from build123d import *

# Parameters (mm, degrees)
SKETCH_1_W                = 192
SKETCH_1_H                = 200
EXTRUDE_1_DEPTH           = 7.5
CHAMFER_1_SIZE            = 1
HOLE_WIZARD_1_D           = 6.6
HOLE_WIZARD_1_CBORE_D     = 11
HOLE_WIZARD_1_CBORE_DEPTH = 6.8
SKETCH_7_R                = 62
CUT_EXTRUDE_1_DEPTH       = 15
HOLE_WIZARD_M6_1_D        = 5


with BuildPart() as part:
    # 草图1 → 凸台-拉伸1 (new, symmetric)
    with BuildSketch(Plane(origin=(0, 0, 0), x_dir=(1, 0, 0), z_dir=(0, 1, 0))):
        Rectangle(SKETCH_1_W, SKETCH_1_H)
    extrude(amount=EXTRUDE_1_DEPTH, both=True)

    # 倒角1
    chamfer_1_edges = [part.edges().sort_by_distance(p)[0] for p in [
        (96, 0, 100),
        (-96, 0, 100),
        (-96, 0, -100),
        (96, 0, -100),
    ]]
    chamfer(chamfer_1_edges, length=CHAMFER_1_SIZE)

    # 打孔尺寸(%根据)内六角圆柱头螺钉的类型1 (through all)
    with Locations(Plane(origin=(0, -7.5, 0), x_dir=(-1, 0, 0), z_dir=(0, -1, 0))):
        with Locations((90, -90), (90, -30), (-90, -30), (-90, -90), (-90, 90), (-90, 30), (90, 30), (90, 90)):
            CounterBoreHole(HOLE_WIZARD_1_D / 2, HOLE_WIZARD_1_CBORE_D / 2, HOLE_WIZARD_1_CBORE_DEPTH)

    # 草图7 → 切除-拉伸1 (cut)
    with BuildSketch(Plane(origin=(0, 7.5, 0), x_dir=(1, 0, 0), z_dir=(0, 1, 0))):
        with Locations(Location((0, 0, 0), (0, 0, 270))):
            Circle(SKETCH_7_R)
    extrude(amount=-CUT_EXTRUDE_1_DEPTH, mode=Mode.SUBTRACT)

    # M6 螺纹孔1 (through all)
    with Locations(Plane(origin=(0, -7.5, 0), x_dir=(-1, 0, 0), z_dir=(0, -1, 0))):
        with Locations((67.5, 0), (62.361868445, -25.831131685), (47.72970773, -47.72970773), (25.831131685, -62.361868445), (0, -67.5), (-25.831131685, -62.361868445), (-47.72970773, -47.72970773), (-62.361868445, -25.831131685), (-67.5, 0), (-62.361868445, 25.831131685), (-47.72970773, 47.72970773), (-25.831131685, 62.361868445), (0, 67.5), (25.831131685, 62.361868445), (47.72970773, 47.72970773), (62.361868445, 25.831131685)):
            Hole(HOLE_WIZARD_M6_1_D / 2)


solid = part.part
Design review of the part built by this model. Coordinates are the model's own, in mm. A direction names the side the tool comes from. Coordinates: 2 decimals unless noted, no trailing zeros. Write each loop counter-clockwise with the first axis right and the second up, starting at its lowest first coordinate (ties: lowest second). Pieces come first, ordered by that corner, then holes. Notation, with made-up numbers: (44, -39.5) - (49, -39.5) arc R20 cw to (49, -19.5) - close; hole circle Ø11 at (32, 55). An arc over 180 degrees is marked (long way). Use one line per item in the form item = value.
Q1. Consider section B-B (z = 90). Write out the cut boundary in (x, y), plus the area to 3 significant figures.
Taken from the geometry:
outline = (-96, -7.5) - (-95.5, -7.5) - (-95.5, -0.7) - (-93.3, -0.7) - (-93.3, 7.5) - (-96, 7.5) - close; (-86.7, -0.7) - (-84.5, -0.7) - (-84.5, -7.5) - (84.5, -7.5) - (84.5, -0.7) - (86.7, -0.7) - (86.7, 7.5) - (-86.7, 7.5) - close; (93.3, -0.7) - (95.5, -0.7) - (95.5, -7.5) - (96, -7.5) - (96, 7.5) - (93.3, 7.5) - close
area = 2,620 mm^2
Q2. The part is to be moulded in two halves that separate along Z. For faces 1 (the flat face through (-1, 0, -100)), 2 (the flat face through (-44, 7.5, -46)), 3 (the cylindrical face through (-45.42, 0.11, -46.77)), say which applies: +Z half, -Z half, draft (parallel to the pull), parting line (faces both ways), or undercut.
Taken from the geometry:
face_1 = -Z half
face_2 = draft
face_3 = undercut
Q3. Insertion check: pin 1 Ø3.5 at (x, z) = (91, -92.5) entering from -Y. The pin has a flat end and moves straight along its axis. Give the tip position at first contact, or say it passes through.
Taken from the geometry:
pin_1 = -0.7
Q4. Consider section D-D (y = -4.75). Count the separate pieces of the cut face and the enclosed holes in it, plus the area to 3 significant figures.
Taken from the geometry:
separate_pieces = 1
enclosed_holes = 25
area = 25,200 mm^2
Q5. Machinability: for faces 4 (the cylindrical face through (94.05, -4.15, -93.72)), 5 (the cylindrical face through (86.7, 3.5, -30.1)), which of the approach directions +Z, -Z, +X, -X, +Y, -Y give a long, thin tool a straight path to every point of the face, cutting with its end or side? Answer none if there is none.
Taken from the geometry:
face_4 = -Y
face_5 = +Y, -Y
Q6. For probe 1 along Z at (x, y) = (-90, 5); probe 2 along X at (y, z) = (0.75, 67.5); probe 3 along X at (y, z) = (-5, -90), list the stretches that pass through material, from the lowest coordinate up.
Taken from the geometry:
probe_1 = -100 to -93.3, -86.7 to -33.3, -26.7 to 26.7, 33.3 to 86.7, 93.3 to 100
probe_2 = -96 to -2.5, 2.5 to 96
probe_3 = -96 to -95.5, -84.5 to 84.5, 95.5 to 96
Q7. Consider section A-A (x = 0). Write out the cut boundary in (y, z), plus the area to 3 significant figures.
Taken from the geometry:
outline = (-7.5, -100) - (7.5, -100) - (7.5, -70) - (-7.5, -70) - close; (-7.5, -65) - (7.5, -65) - (7.5, -62) - (-7.5, -62) - close; (-7.5, 62) - (7.5, 62) - (7.5, 65) - (-7.5, 65) - close; (-7.5, 70) - (7.5, 70) - (7.5, 100) - (-7.5, 100) - close
area = 990 mm^2
Q8. Consider section C-C (x = -67.5). Write out the cut boundary in (y, z).
Taken from the geometry:
outline = (-7.5, -100) - (7.5, -100) - (7.5, -2.5) - (-7.5, -2.5) - close; (-7.5, 2.5) - (7.5, 2.5) - (7.5, 100) - (-7.5, 100) - close
